The model under review builds one solid part; all positions refer to its coordinate system, in mm. A direction names the side the tool comes from. Give positions to 0.01 mm unless a question says otherwise; leave off trailing zeros. Loops run counter-clockwise (first coordinate to the right, second up) from the corner with the lowest first, then second, coordinate; pieces in that order, holes last. Notation, with made-up numbers: (33, 41) - (63, 41) arc R29 ccw to (63, 67) - close; hole circle Ø3 at (-7.75, -8.5). An arc over 180 degrees is marked (long way). Answer as a JSON object with one key per item and string values.
from build123d import *

# Parameters (mm, degrees)
SKETCH_1_W          = 225
SKETCH_1_H          = 76
EXTRUDE_1_DEPTH     = 80
SKETCH_2_W          = 75
SKETCH_2_H          = 76
CUT_EXTRUDE_1_DEPTH = 90
SKETCH_3_W          = 75
SKETCH_3_H          = 76
CUT_EXTRUDE_2_DEPTH = 15
SKETCH_4_R          = 2.5
CUT_EXTRUDE_3_DEPTH = 15
SKETCH_5_R          = 35
EXTRUDE_2_DEPTH     = 79
SKETCH_6_R          = 12.5
EXTRUDE_3_DEPTH     = 19
SKETCH_7_W          = 105
SKETCH_7_H          = 35
CUT_EXTRUDE_4_DEPTH = 19
EXTRUDE_4_DEPTH     = 8


with BuildPart() as part:
    # 草图1 → 凸台-拉伸1 (new body)
    with BuildSketch(Plane.XY):
        Rectangle(SKETCH_1_W, SKETCH_1_H)
    extrude(amount=EXTRUDE_1_DEPTH)

    # 草图2 → 切除-拉伸1 (cut)
    with BuildSketch(Plane.ZY.offset(112.5)):
        with Locations((37.5, 0)):
            Rectangle(SKETCH_2_W, SKETCH_2_H)
    extrude(amount=-CUT_EXTRUDE_1_DEPTH, mode=Mode.SUBTRACT)

    # 草图3 → 切除-拉伸2 (cut)
    with BuildSketch(Plane(origin=(112.5, 0, 0), x_dir=(0, 0, -1), z_dir=(1, 0, 0))):
        with Locations((-37.5, 0)):
            Rectangle(SKETCH_3_W, SKETCH_3_H)
    extrude(amount=-CUT_EXTRUDE_2_DEPTH, mode=Mode.SUBTRACT)

    # 草图4 → 切除-拉伸3 (cut)
    with BuildSketch(Plane(origin=(0, 0, 75), x_dir=(-1, 0, 0), z_dir=(0, 0, -1))):
        with Locations((104, -25)):
            Circle(SKETCH_4_R)
        with Locations((104, 25)):
            Circle(SKETCH_4_R)
        with Locations((-104, -25)):
            Circle(SKETCH_4_R)
        with Locations((-104, 25)):
            Circle(SKETCH_4_R)
    extrude(amount=-CUT_EXTRUDE_3_DEPTH, mode=Mode.SUBTRACT)

    # 草图5 → 凸台-拉伸2 (add)
    with BuildSketch(Plane.ZY.offset(22.5)):
        with Locations(Location((37.5, 0, 0), (0, 0, 180))):
            Circle(SKETCH_5_R)
    extrude(amount=EXTRUDE_2_DEPTH)

    # 草图6 → 凸台-拉伸3 (add)
    with BuildSketch(Plane.ZY.offset(101.5)):
        with Locations((37.5, 0)):
            Circle(SKETCH_6_R)
    extrude(amount=EXTRUDE_3_DEPTH)

    # 草图7 → 切除-拉伸4 (cut)
    with BuildSketch(Plane.XY.offset(80)):
        with Locations((42, -18.5)):
            Rectangle(SKETCH_7_W, SKETCH_7_H)
    extrude(amount=-CUT_EXTRUDE_4_DEPTH, mode=Mode.SUBTRACT)

    # 草图8 → 凸台-拉伸4 (add)
    with BuildSketch(Plane(origin=(97.5, 0, 0), x_dir=(0, 0, -1), z_dir=(1, 0, 0))):
        Polygon((-75, 38), (0, 38), (0, -38), (-75, -38), (-75, -36), (-2, -36), (-2, 36), (-75, 36), align=None)
    extrude(amount=EXTRUDE_4_DEPTH)


solid = part.part
Q1. Consider section C-C, the plane y = 25. State the section outline as (x, z) points, plus the area to 3 significant figures.
Results:
{"outline": "(-112.5, 75) - (-106.5, 75) - (-106.5, 80) - (-112.5, 80) - close; (-101.5, 13.01) - (-22.5, 13.01) - (-22.5, 0) - (105.5, 0) - (105.5, 2) - (97.5, 2) - (97.5, 75) - (101.5, 75) - (101.5, 80) - (-101.5, 80) - (-101.5, 75) - (-22.5, 75) - (-22.5, 61.99) - (-101.5, 61.99) - close; (106.5, 75) - (112.5, 75) - (112.5, 80) - (106.5, 80) - close", "area": "14,000 mm^2"}
Q2. Clearance check with flat-ended pins moving along their axes: pin 1 Ø4 at (x, y) = (-64.5, -19.5) entering from -Z; pin 2 Ø3 at (y, z) = (-6, 43) entering from +X; pin 3 Ø8 at (x, y) = (-34, 30) entering from -Z; pin 4 Ø6.5 at (x, y) = (-104, -25) entering from +Z. State where each tip first meets the part, or that it passes through.
Results:
{"pin 1": "stops at z = 7.19", "pin 2": "stops at x = 97.5", "pin 3": "stops at z = 14.07", "pin 4": "stops at z = 80"}
Q3. Consider section D-D, the plane z = 37.5. State the section outline as (x, y) points, plus the area to 3 significant figures.
Results:
{"outline": "(-120.5, -12.5) - (-101.5, -12.5) - (-101.5, -35) - (-22.5, -35) - (-22.5, -38) - (105.5, -38) - (105.5, -36) - (97.5, -36) - (97.5, 36) - (105.5, 36) - (105.5, 38) - (-22.5, 38) - (-22.5, 35) - (-101.5, 35) - (-101.5, 12.5) - (-120.5, 12.5) - close", "area": "15,200 mm^2"}
Q4. The part is to be moulded in two halves that separate along Y. For faces 1 (the face through (48, 38, 41)), 2 (the face through (-106.385, 25.751, 77.465)), 3 (the face through (-2, 9, 80)), 4 (the face through (105, -1, 75)), say which applies: +Y half, -Y half, draft (parallel to the pull), parting line (faces both ways), or undercut.
Results:
{"face 1": "+Y half", "face 2": "undercut", "face 3": "draft", "face 4": "undercut"}
Q5. To check wall thickness, follow probe 1 along Y at (x, z) = (-104, 78.7); probe 2 along X at (y, z) = (-22.5, 70.5); probe 3 along X at (y, z) = (-16, 53.5). State the ranges of each line that lie inside material, in increasing order. Write a range as [from, to].
Results:
{"probe 1": "y = [-38, -27.5], [-22.5, 22.5], [27.5, 38]", "probe 2": "x = [-22.5, -10.5], [94.5, 97.5]", "probe 3": "x = [-101.5, 97.5]"}
Q6. Consider section A-A, the plane x = -46. State the section outline as (y, z) points.
Results:
{"outline": "(-38, 75) - (38, 75) - (38, 80) - (-38, 80) - close; circle Ø70 at (0, 37.5)"}
Q7. Consider section B-B, the plane x = -104. State the section outline as (y, z) points.
Results:
{"outline": "(-38, 75) - (-27.5, 75) - (-27.5, 80) - (-38, 80) - close; (-22.5, 75) - (22.5, 75) - (22.5, 80) - (-22.5, 80) - close; circle Ø25 at (0, 37.5); (27.5, 75) - (38, 75) - (38, 80) - (27.5, 80) - close"}
Q8. For faces 5 (the face through (101, -1, 2)), 6 (the face through (-68, -1, 75)), 7 (the face through (105.5, 0, 1)), 8 (the face through (-10.5, -19, 71)), list the 3-axis set-ups (+Z, -Z, +X, -X, +Y, -Y) from which the entire face can be reached by the end or side of a thin tool; tool diameter is ignored.
Results:
{"face 5": "+X", "face 6": "-X, +Y, -Y", "face 7": "-Z, +X, +Y, -Y", "face 8": "+Z"}
